```python
from build123d import *

# Parameters (mm, degrees)
SKETCH1_W                                           = 420
SKETCH1_H                                           = 22
BOSS_EXTRUDE1_DEPTH                                 = 27
SKETCH2_W                                           = 420
SKETCH2_H                                           = 2
BOSS_EXTRUDE2_DEPTH                                 = 2
M5_TAPPED_HOLE1_D                                   = 4.2
M5_TAPPED_HOLE1_DEPTH                               = 12.4
M5_TAPPED_HOLE1_TIP                                 = 1.2618073
CBORE_FOR_M5_HEX_SOCKET_HEAD_CAP_SCREW1_D           = 5.5
CBORE_FOR_M5_HEX_SOCKET_HEAD_CAP_SCREW1_CBORE_D     = 10
CBORE_FOR_M5_HEX_SOCKET_HEAD_CAP_SCREW1_CBORE_DEPTH = 17


with BuildPart() as part:
    # Sketch1 → Boss-Extrude1 (new body)
    with BuildSketch(Plane.XY):
        Rectangle(SKETCH1_W, SKETCH1_H)
    extrude(amount=BOSS_EXTRUDE1_DEPTH)

    # Sketch2 → Boss-Extrude2 (add)
    with BuildSketch(Plane.XY.offset(27)):
        with Locations((0, 10)):
            Rectangle(SKETCH2_W, SKETCH2_H)
    extrude(amount=BOSS_EXTRUDE2_DEPTH)

    # M5 Tapped Hole1
    with Locations(Plane.XY.offset(27)):
        with Locations((180, -1), (120, -1), (60, -1), (0, -1), (-180, -1), (-120, -1), (-60, -1)):
            Hole(M5_TAPPED_HOLE1_D / 2, depth=M5_TAPPED_HOLE1_DEPTH)
            with Locations((0, 0, -(M5_TAPPED_HOLE1_DEPTH + M5_TAPPED_HOLE1_TIP / 2))):  # 118° drill point
                Cone(0, M5_TAPPED_HOLE1_D / 2, M5_TAPPED_HOLE1_TIP, mode=Mode.SUBTRACT)

    # CBORE for M5 Hex Socket Head Cap Screw1 (through all)
    with Locations(Plane.XY.offset(27)):
        with Locations((200, 0), (80, 0), (-80, 0), (-200, 0)):
            CounterBoreHole(CBORE_FOR_M5_HEX_SOCKET_HEAD_CAP_SCREW1_D / 2, CBORE_FOR_M5_HEX_SOCKET_HEAD_CAP_SCREW1_CBORE_D / 2, CBORE_FOR_M5_HEX_SOCKET_HEAD_CAP_SCREW1_CBORE_DEPTH)


solid = part.part
```
For this review, take the finished solid that the model builds, in its own axes (mm). A direction names the side the tool comes from. Round coordinates to 2 decimals unless told otherwise and drop trailing zeros. Write each loop counter-clockwise with the first axis right and the second up, starting at its lowest first coordinate (ties: lowest second). Pieces come first, ordered by that corner, then holes. Notation, with made-up numbers: M -8,42.5 L 3,42.5 A25 ccw 3,78.5 Z; hole C 3.25,58.25 d8. An arc over 180 degrees is marked long. One line per item, written item: value. Start each with the question number.
(1) The part is to be moulded in two halves that separate along X. For faces 1 (the flat face through (-210, 0, 14)), 2 (the flat face through (-197.8, -2.2, 10)), 3 (the cylindrical face through (84.619, -1.915, 18.619)), 4 (the flat face through (-3, 0, 0)), say which applies: released by +X, released by -X, zero draft, split by the parting line, or undercut.
(2) Wall thickness on line 1 (Y direction, x = -80, z = 20); line 2 (X direction, y = 3.25, z = 19); line 3 (X direction, y = 4.5, z = 17): over which ranges is each line inside the solid? List them lowest first.
(3) Machinability: for faces 5 (the cylindrical face through (-75.381, -1.915, 18.619)), 6 (the flat face through (-3, -11, 13)), 7 (the flat face through (-3, -1, 27)), which of the approach directions +Z, -Z, +X, -X, +Y, -Y give a long, thin tool a straight path to every point of the face, cutting with its end or side? Answer none if there is none.
(4) We need section B-B (x = 29). Give the boundary of the cut face in (y, z).
(5) We need section A-A (z = 18). Count the separate pieces of the cut face and the enclosed holes in it, and give its area (3 significant figures).
(6) Insertion check: pin 1 (5.5 mm diameter, centred on x = 120, y = -1, fed in from +Z); pin 2 (4.5 mm diameter, centred on x = 200, y = 0, fed in from +Z); pin 3 (2.5 mm diameter, centred on x = 60, y = -1, fed in from +Z); pin 4 (8 mm diameter, centred on x = 80, y = 0, fed in from +Z). Each pin has a flat end and moves straight along its axis. Give the tip position at first contact, or say it passes through.
Result:
1. face 1: released by -X
1. face 2: undercut
1. face 3: undercut
1. face 4: zero draft
2. line 1: -11 to -5, 5 to 11
2. line 2: -210 to -203.8, -196.2 to -83.8, -76.2 to 76.2, 83.8 to 196.2, 203.8 to 210
2. line 3: -210 to -202.18, -197.82 to -82.18, -77.82 to 77.82, 82.18 to 197.82, 202.18 to 210
3. face 5: +Z
3. face 6: +Z, -Z, +X, -X, -Y
3. face 7: +Z, +X, -X, -Y
4. outline: M -11,0 L 11,0 L 11,29 L 9,29 L 9,27 L -11,27 Z
5. separate pieces: 1
5. enclosed holes: 11
5. area: 8,830 mm²
6. pin 1: z = 27
6. pin 2: through
6. pin 3: z = 14.09
6. pin 4: z = 10
